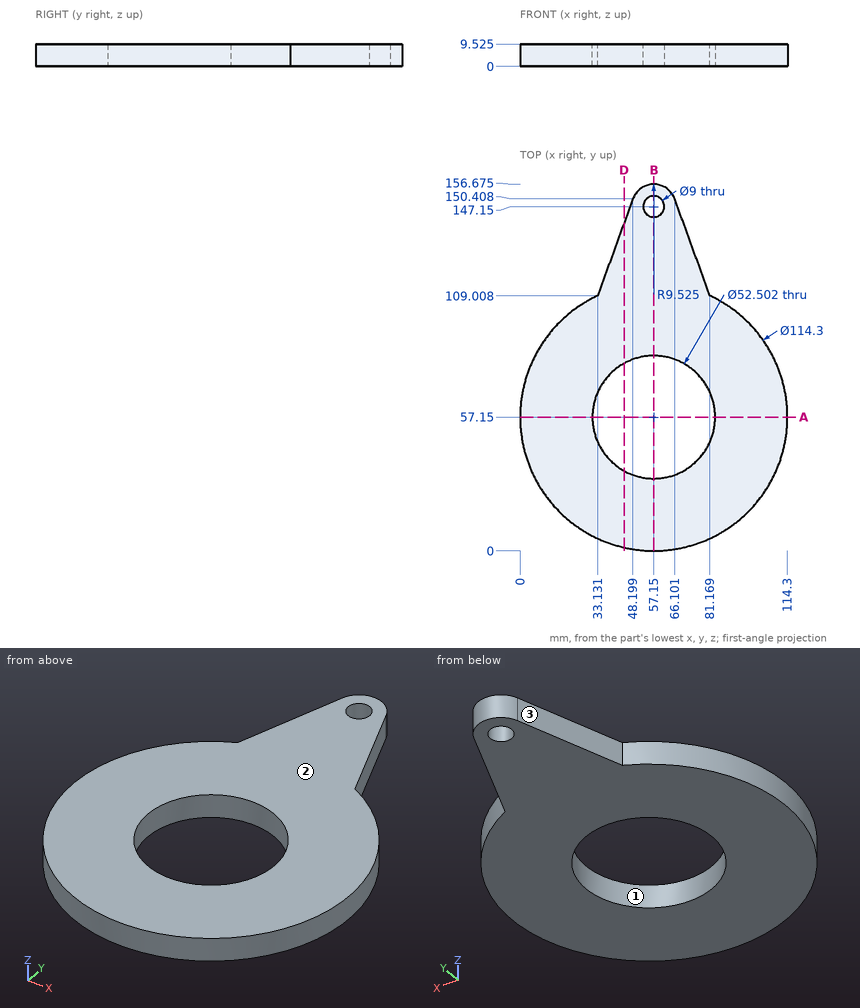
The drawing under review shows one solid part. Ordinate dimensions are in mm from its lowest x, y, z. Round coordinates to 2 decimals unless told otherwise and drop trailing zeros. Loops run counter-clockwise (first coordinate to the right, second up) from the corner with the lowest first, then second, coordinate; pieces in that order, holes last. Notation, with made-up numbers: (64.25, 72.25) - (72.25, 72.25) arc R8 cw to (72.25, 81.25) - close; hole circle Ø5 at (-11, 40.5). An arc over 180 degrees is marked (long way). One line per item, written item: value. Start each with the question number.
1) Consider section D-D on x = 44.5. Give the boundary of the cut face in (y, z) (1 decimal).
2) To check wall thickness, follow L1, parallel to X at y = 57.15, z = 6; L2, parallel to X at y = 35, z = 8.75 (1 decimal); L3, parallel to X at y = 105, z = 8.75. State the ranges of each line that lie inside material, in increasing order. Write a range as from..to.
3) Consider section B-B on x = 57.15. Give the number of separate pieces and of enclosed holes in the cut face.
4) Consider section A-A on y = 57.15. Give the boundary of the cut face in (x, z) (1 decimal).
5) Draft analysis for pull direction Y (two halves, no side actions). For the marked faces 1, 2 and 3, state which applies: +Y half, -Y half, draft (parallel to the pull), parting line (faces both ways), or undercut.
6) Insertion check: pin 1 Ø10 at (x, y) = (41, 80) entering from -Z; pin 2 Ø5 at (y, z) = (46, 5) entering from -X. Each pin has a flat end and moves straight along its axis. Give the tip position at first contact, or say it passes through.
Reported:
1. outline: (1.4, 0) - (34.1, 0) - (34.1, 9.5) - (1.4, 9.5) - close; (80.2, 0) - (140.2, 0) - (140.2, 9.5) - (80.2, 9.5) - close
2. L1: x = 0..30.9, 83.4..114.3
2. L2: x = 4.5..43.1, 71.2..109.8
2. L3: x = 25.9..88.4
3. separate pieces: 3
3. enclosed holes: 0
4. outline: (0, 0) - (30.9, 0) - (30.9, 9.5) - (0, 9.5) - close; (83.4, 0) - (114.3, 0) - (114.3, 9.5) - (83.4, 9.5) - close
5. face 1: undercut
5. face 2: draft
5. face 3: +Y half
6. pin 1: stops at z = 0
6. pin 2: stops at x = 0.66
